Here's how the part is built. I have some questions about the finished solid (model axes, mm). A direction names the side the tool comes from. Round coordinates to 2 decimals unless told otherwise and drop trailing zeros. Order: outer loops, then holes, each group sorted by start corner. A loop starts at its lowest first (then second) coordinate and runs counter-clockwise, first axis right, second up.
```python
from build123d import *

# Parameters (mm, degrees)
BOSS_EXTRUDE1_DEPTH = 12.7


with BuildPart() as part:
    # Sketch1 → Boss-Extrude1 (new, symmetric)
    with BuildSketch(Plane.XY):
        with BuildLine():
            Line((57.15, 0), (57.15, 4.7625))
            Line((57.15, 4.7625), (44.45, 4.7625))
            ThreePointArc((44.45, 4.7625), (38.837339924, 7.087339924), (36.5125, 12.7))
            ThreePointArc((36.5125, 12.7), (0, 49.2125), (-36.5125, 12.7))
            ThreePointArc((-36.5125, 12.7), (-38.837339924, 7.087339924), (-44.45, 4.7625))
            Line((-44.45, 4.7625), (-57.15, 4.7625))
            Line((-57.15, 4.7625), (-57.15, 0))
            Line((-57.15, 0), (-44.45, 0))
            ThreePointArc((-44.45, 0), (-35.469743879, 3.719743879), (-31.75, 12.7))
            ThreePointArc((-31.75, 12.7), (0, 44.45), (31.75, 12.7))
            ThreePointArc((31.75, 12.7), (35.469743879, 3.719743879), (44.45, 0))
            Line((44.45, 0), (57.15, 0))
        make_face()
    extrude(amount=BOSS_EXTRUDE1_DEPTH, both=True)


solid = part.part
```
1) I'm going to push flat-ended pins straight in: pin 1 (3 mm diameter, centred on x = 34, z = 2.5, fed in from -Y); pin 2 (1.5 mm diameter, centred on y = 44, z = -7.5, fed in from -X); pin 3 (4 mm diameter, centred on y = 16, z = 1.5, fed in from -X). Where does each tip first touch, or does it pass through?
2) If we section it at B-B (y = 25.5): Write out the boundary of the cut face in (x, z), plus the area to 3 significant figures.
3) If we section it at D-D (y = 35.5): Write out the boundary of the cut face in (x, z), plus the area to 3 significant figures.
4) I need wall thicknesses on line 1 (X direction, y = 12.5, z = 8.5); line 2 (X direction, y = 13, z = 0); line 3 (Y direction, x = 28, z = 8.75). Which ranges of each line are inside material? Lowest first, please.
5) If we section it at C-C (x = 0): Write out the boundary of the cut face in (y, z).
6) For faces 5 (the flat face through (-51, 4.762, 0)), 6 (the cylindrical face through (-35.57, 3.62, 0.18)), 7 (the flat face through (51, 4.762, 0)), 8 (the flat face through (0, 45, 12.7)), which set-ups out of +Z, -Z, +X, -X, +Y, -Y let a thin tool reach every point of the face, with its end or its side?
7) We'd pull the mould along X, two halves only. Please class faces 1 (the cylindrical face through (-38.776, 7.149, 0.178)), 2 (the flat face through (-51, 0, 0)), 3 (the cylindrical face through (38.899, 7.026, 0.178)), 4 (the cylindrical face through (35.37, 3.82, 0.18)): +X half, -X half, draft (parallel to the pull), parting line (faces both ways), or undercut.
Solutions:
1. pin 1: stops at y = 3.69
1. pin 2: stops at x = -20
1. pin 3: stops at x = -36.49
2. outline: (-34.2, -12.7) - (-29.06, -12.7) - (-29.06, 12.7) - (-34.2, 12.7) - close; (29.06, -12.7) - (34.2, -12.7) - (34.2, 12.7) - (29.06, 12.7) - close
2. area: 261 mm2
3. outline: (-28.52, -12.7) - (-22.1, -12.7) - (-22.1, 12.7) - (-28.52, 12.7) - close; (22.1, -12.7) - (28.52, -12.7) - (28.52, 12.7) - (22.1, 12.7) - close
3. area: 326 mm2
4. line 1: x = -36.52 to -31.75, 31.75 to 36.52
4. line 2: x = -36.51 to -31.75, 31.75 to 36.51
4. line 3: y = 27.67 to 36.13
5. outline: (44.45, -12.7) - (49.21, -12.7) - (49.21, 12.7) - (44.45, 12.7) - close
6. face 5: +Z, -Z, -X, +Y
6. face 6: +Z, -Z, -Y
6. face 7: +Z, -Z, +X, +Y
6. face 8: +Z, +X, -X, +Y, -Y
7. face 1: -X half
7. face 2: draft
7. face 3: +X half
7. face 4: undercut
